from build123d import *

# Parameters (mm, degrees)
EXTRUDE_START       = -3
SKETCH_2_R          = 35.459459581
EXTRUDE_1_DEPTH     = 3
SKETCH_4_R          = 3
CUT_EXTRUDE_1_DEPTH = 59.532042507


with BuildPart() as part:
    # 草图1 → 旋转1 (revolve)
    with BuildSketch(Plane(origin=(0, 0, 0), x_dir=(0, 0, -1), z_dir=(1, 0, 0)), mode=Mode.PRIVATE) as revolve_1_sk:
        with BuildLine():
            Line((0, 12), (23.23298563, 12))
            ThreePointArc((23.23298563, 12), (27.23298563, 10.92820323), (30.16118886, 8))
            Line((30.16118886, 8), (41, 8))
            Line((41, 8), (41, 5))
            Line((41, 5), (31, 5))
            Line((31, 5), (31, 0))
            Line((31, 0), (28, 0))
            Line((28, 0), (27.172216642, 4.694592711))
            ThreePointArc((27.172216642, 4.694592711), (25.804136068, 7.064177772), (23.23298563, 8))
            Line((23.23298563, 8), (21.200995797, 8))
            Line((21.200995797, 8), (0, 8))
            Line((0, 8), (0, 12))
        make_face()
    revolve(revolve_1_sk.sketch.rotate(Axis((0, 53.940866142, 0), (0, -1, 0)), 180), axis=Axis((0, 53.940866142, 0), (0, -1, 0)))

    # 草图2 → 凸台-拉伸1 (add)
    with BuildSketch(Plane(origin=(0, 8, 0), x_dir=(1, 0, 0), z_dir=(0, 1, 0)).offset(EXTRUDE_START)):
        with BuildLine():
            Line((-34.294678434, 23.688076669), (-33.80549374, 23.198892063))
            ThreePointArc((-33.80549374, 23.198892063), (-40.999999826, -0.003774812), (-33.801221389, -23.205116518))
            Line((-33.801221389, -23.205116518), (-34.233536486, -23.627631697))
            ThreePointArc((-34.233536486, -23.627631697), (-34.294678888, -34.294678888), (-23.627631697, -34.233536486))
            Line((-23.627631697, -34.233536486), (-23.205116518, -33.801221389))
            ThreePointArc((-23.205116518, -33.801221389), (-0.003771108, -40.999999827), (23.198898172, -33.805489549))
            Line((23.198898172, -33.805489549), (23.680662822, -34.287254142))
            ThreePointArc((23.680662822, -34.287254142), (34.291151869, -34.298203544), (34.294310993, -23.687709319))
            Line((34.294310993, -23.687709319), (33.805466141, -23.198932281))
            ThreePointArc((33.805466141, -23.198932281), (40.997262845, 0.473750181), (33.260352966, 23.973921676))
            Line((33.260352966, 23.973921676), (33.682868145, 24.406236773))
            ThreePointArc((33.682868145, 24.406236773), (33.629998505, 33.629998505), (24.406236773, 33.682868145))
            Line((24.406236773, 33.682868145), (23.973921676, 33.260352966))
            ThreePointArc((23.973921676, 33.260352966), (0.470906346, 40.997295609), (-23.203621987, 33.802247362))
            Line((-23.203621987, 33.802247362), (-23.642860481, 34.249073393))
            ThreePointArc((-23.642860481, 34.249073393), (-34.27192479, 34.317335821), (-34.294678434, 23.688076669))
        make_face()
        Circle(SKETCH_2_R, mode=Mode.SUBTRACT)
    extrude(amount=EXTRUDE_1_DEPTH)

    # 草图4 → 切除-拉伸1 (cut, through all)
    with BuildSketch(Plane(origin=(0, 8, 0), x_dir=(1, 0, 0), z_dir=(0, 1, 0))):
        with Locations(Location((-28.991378029, 28.991378029, 0), (0, 0, 270))):
            Circle(SKETCH_4_R)
        with Locations(Location((28.991378029, 28.991378029, 0), (0, 0, 270))):
            Circle(SKETCH_4_R)
        with Locations(Location((28.991378029, -28.991378029, 0), (0, 0, 270))):
            Circle(SKETCH_4_R)
        with Locations(Location((-28.991378029, -28.991378029, 0), (0, 0, 270))):
            Circle(SKETCH_4_R)
    extrude(amount=-CUT_EXTRUDE_1_DEPTH, mode=Mode.SUBTRACT)


solid = part.part
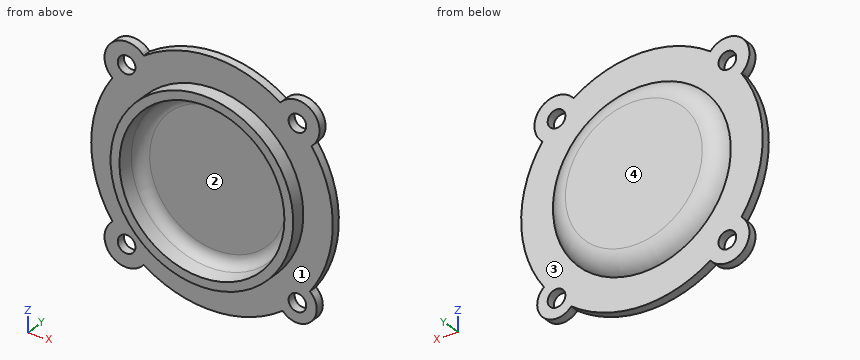
Source: CAD feature listing. Evaluate the final solid. Frame: model axes, mm. Face numbers are marked on the shaded views. A direction names the side the tool comes from. Round coordinates to 2 decimals unless told otherwise and drop trailing zeros. Loops run counter-clockwise (first coordinate to the right, second up) from the corner with the lowest first, then second, coordinate; pieces in that order, holes last.
Q1. Section A-A, the plane z = 0. Return loops of the section in (x, y), plus the area to 3 significant figures.
Q2. Section B-B, the plane x = 0. Return loops of the section in (y, z), plus the area to 3 significant figures.
Q3. Access query for the marked faces 3 and 4. Directions: +Z, -Z, +X, -X, +Y, -Y. A direction counts if a zero-diameter tool reaches every point of the face in a straight line with its end or side. Return the directions, or none.
Q4. Section C-C, the plane y = 3.5. Return loops of the section in (x, z).
Q5. First-contact query: P1, Ø5, axis at x = -32.5, z = -10.5, coming from the -Y side; P2, Ø7, axis at x = -28.99, z = -28.99, coming from the +Y side; P3, Ø3, axis at y = 1.5, z = -26, coming from the +X side; P4, Ø5.5, axis at x = -28.99, z = 28.99, coming from the +Y side. Flat tips, straight axial feed; report the tip coordinate or a pass-through.
Q6. Mould query, pull axis Z, two halves, no side actions, for the marked faces 1 and 2. Classes: pulls with the +Z half, pulls with the -Z half, needs draft (parallel to the pull), parting line crosses it, or undercut.
Q7. Ray query, line 1 (Y direction, x = 5.5, z = -18); line 2 (Y direction, x = 30, z = -14.5); line 3 (Z direction, x = 18.5, y = 7). Return the intervals inside material, ascending.
Solutions:
1. outline: (-41, 5) - (-31, 5) - (-31, 0) - (-28, 0) - (-27.17, 4.69) arc R4 cw to (-23.23, 8) - (23.23, 8) arc R4 cw to (27.17, 4.69) - (28, 0) - (31, 0) - (31, 5) - (41, 5) - (41, 8) - (30.16, 8) arc R8 ccw to (23.23, 12) - (-23.23, 12) arc R8 ccw to (-30.16, 8) - (-41, 8) - close
1. area: 349 mm2
2. outline: (0, -31) - (5, -31) - (5, -41) - (8, -41) - (8, -30.16) arc R8 ccw to (12, -23.23) - (12, 23.23) arc R8 ccw to (8, 30.16) - (8, 41) - (5, 41) - (5, 31) - (0, 31) - (0, 28) - (4.69, 27.17) arc R4 cw to (8, 23.23) - (8, -23.23) arc R4 cw to (4.69, -27.17) - (0, -28) - close
2. area: 349 mm2
3. face 3: +Y
3. face 4: +Z, -Z, +X, -X, +Y
4. outline: circle Ø62 at (0, 0); hole circle Ø54.77 at (0, 0)
5. P1: stops at y = 5
5. P2: stops at y = 8
5. P3: stops at x = 18.99
5. P4: passes through
6. face 1: needs draft
6. face 2: undercut
7. line 1: y = 8 to 12
7. line 2: y = 5 to 8
7. line 3: z = -36.59 to -18.1, 18.1 to 36.59
